from build123d import *

# Parameters (mm, degrees)
CUT_EXTRUDE1_DEPTH = 3


with BuildPart() as part:
    # Logo3_bib1 → Revolve1 (revolve)
    with BuildSketch(Plane(origin=(0, 0, 0), x_dir=(-1, 0, 0), z_dir=(0, -1, 0))):
        with BuildLine():
            Line((0, -22), (0, 8))
            Line((0, 8), (6, 8))
            ThreePointArc((6, 8), (6.353553391, 7.853553391), (6.5, 7.5))
            Line((6.5, 7.5), (6.5, 0))
            Line((6.5, 0), (4, 0))
            Line((4, 0), (4, -0.01))
            Line((4, -0.01), (3.488425636, -0.01))
            ThreePointArc((3.488425636, -0.01), (3.468729481, -0.026527036), (3.481585234, -0.048793852))
            Line((3.481585234, -0.048793852), (4, -0.237481396))
            Line((4, -0.237481396), (4, -21.375))
            Line((4, -21.375), (3.375, -22))
            Line((3.375, -22), (0, -22))
        make_face()
    revolve(axis=Axis((0, 0, -10.585154653), (0, 0, 1)))

    # Logo3_bib2 → Cut-Extrude1 (cut)
    with BuildSketch(Plane(origin=(0, 0, -8), x_dir=(1, 0, 0), z_dir=(0, 0, -1))):
        Polygon((3.464101615, 0), (1.732050808, 3), (-1.732050808, 3), (-3.464101615, 0), (-1.732050808, -3), (1.732050808, -3), align=None)
    extrude(amount=-CUT_EXTRUDE1_DEPTH, mode=Mode.SUBTRACT)


solid = part.part
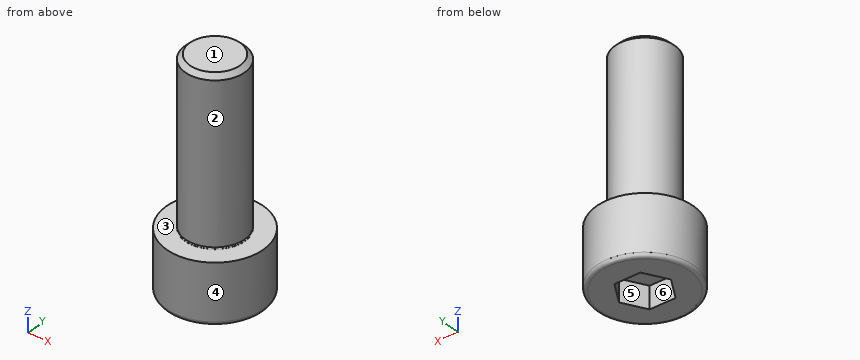
Geometry: final body of the model. Coordinates: model frame, mm. Face numbers are marked on the shaded views. A direction names the side the tool comes from. Coordinates: 2 decimals unless noted, no trailing zeros. Loops run counter-clockwise (first coordinate to the right, second up) from the corner with the lowest first, then second, coordinate; pieces in that order, holes last. Notation, with made-up numbers: (-33.75, 65) - (-8.75, 65) arc R22 ccw to (-8.75, 84) - close; hole circle Ø7 at (28, -2.75). An arc over 180 degrees is marked (long way). One line per question, with ' | ' between items. Start each with the question number.
(1) Cut plane A-A on x = 0. Output: boundary loops of the cut face in (y, z) (3 decimals), and give its area (3 significant figures).
(2) Cut plane B-B on z = 11. Output: boundary loops of the cut face in (x, y), and give its area (3 significant figures).
(3) Draft query along Y for the marked faces 3, 4, 5 and 6. Return one class per face: +Y half, -Y half, draft (parallel to the pull), parting line (faces both ways), or undercut.
(4) Ray query, L1, parallel to Y at x = -2, z = 13; L2, parallel to Z at x = -1.5, y = 4.5; L3, parallel to X at y = 2.25, z = -6. Return the intervals inside material, ascending. Write a range as from..to.
(5) Reachability of the marked faces 1 and 2 from +Z, -Z, +X, -X, +Y, -Y: full face, straight path, thin tool, end or side. Return the list, or none.
(6) First-contact query: pin 1 (1.8 mm diameter, centred on x = -1.5, y = 0, fed in from -Z); pin 2 (6 mm diameter, centred on y = 5, z = 7, fed in from +X); pin 3 (5 mm diameter, centred on x = 2.5, z = 10, fed in from -Y). Flat tips, straight axial feed; report the tip coordinate or a pass-through.
Here are the results:
1) outline: (-6.5, -7.5) arc R0.5 ccw to (-6, -8) - (-3, -8) - (-3, -5) - (3, -5) - (3, -8) - (6, -8) arc R0.5 ccw to (6.5, -7.5) - (6.5, 0) - (4, 0) - (4, 0.01) - (3.488, 0.01) arc R0.02 cw to (3.482, 0.049) - (4, 0.237) - (4, 21.375) - (3.375, 22) - (-3.375, 22) - (-4, 21.375) - (-4, 0.237) - (-3.482, 0.049) arc R0.02 cw to (-3.488, 0.01) - (-4, 0.01) - (-4, 0) - (-6.5, 0) - close | area: 261 mm²
2) outline: circle Ø8 at (0, 0) | area: 50.3 mm²
3) face 3: draft | face 4: parting line | face 5: undercut | face 6: undercut
4) L1: -3.46..3.46 | L2: -8..0 | L3: -6.1..-2.17, 2.17..6.1
5) face 1: +Z, +X, -X, +Y, -Y | face 2: +Z
6) pin 1: z = -5 | pin 2: x = 3.46 | pin 3: y = -4
